For this review, take the finished solid that the model builds, in its own axes (mm). Coordinates: 2 decimals unless noted, no trailing zeros. Order: outer loops, then holes, each group sorted by start corner. A loop starts at its lowest first (then second) coordinate and runs counter-clockwise, first axis right, second up. Notation, with made-up numbers: (68, 72) -> (110, 72) arc R32 cw to (110, 105) -> close; hole circle Ø6 at (30, 80.25). An arc over 180 degrees is marked (long way). Answer as a JSON object with one key per item and string values. Group by question number.
1) Add section C-C, the plane y = -85. Write out the cut boundary in (x, z).
2) Add section A-A, the plane x = 75. Write out the cut boundary in (y, z), then the cut area to 3 significant figures.
3) Wall thickness on L1, parallel to Y at x = -75, z = -2.25; L2, parallel to X at y = -87.5, z = -1.25; L3, parallel to Y at x = 76.5, z = 4.75: over which ranges is each line inside the solid? List them lowest first.
4) For pin 1 (18 mm diameter, centred on x = 75, y = -85, fed in from +Z), flat-tipped, find the tip position at first contact; note if it passes through.
5) Add section B-B, the plane z = -4.5. Write out the cut boundary in (x, y).
from build123d import *

# Parameters (mm, degrees)
SKETCH1_W           = 250
SKETCH1_H           = 220
BOSS_EXTRUDE1_DEPTH = 8
F_14_HOLE1_D        = 14
FILLET2_R           = 20


with BuildPart() as part:
    # Sketch1 → Boss-Extrude1 (new, symmetric)
    with BuildSketch(Plane.XY):
        Rectangle(SKETCH1_W, SKETCH1_H)
    extrude(amount=BOSS_EXTRUDE1_DEPTH, both=True)

    # Ø14 Hole1 (through all)
    with Locations(Plane.XY.offset(8)):
        with Locations((-75, 85), (75, 85), (75, -85), (-75, -85)):
            Hole(F_14_HOLE1_D / 2)

    # Fillet2
    fillet2_edges = [part.edges().sort_by_distance(p)[0] for p in [
        (-125, 110, 0),
        (125, 110, 0),
        (125, -110, 0),
        (-125, -110, 0),
    ]]
    fillet(fillet2_edges, radius=FILLET2_R)


solid = part.part
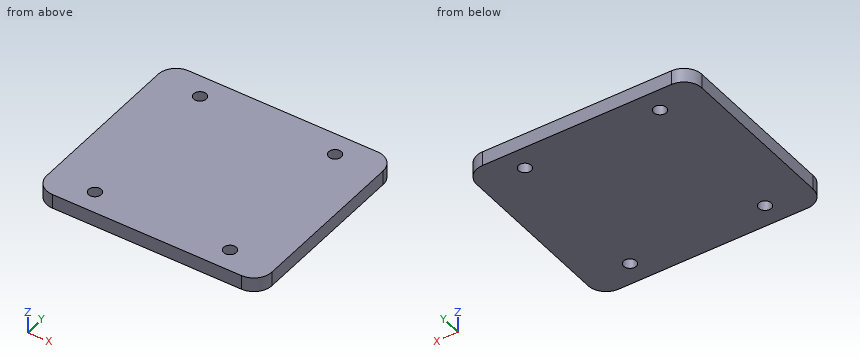
Output values:
{
 "1": {"outline": "(-125, -8) -> (-82, -8) -> (-82, 8) -> (-125, 8) -> close; (-68, -8) -> (68, -8) -> (68, 8) -> (-68, 8) -> close; (82, -8) -> (125, -8) -> (125, 8) -> (82, 8) -> close"},
 "2": {"outline": "(-110, -8) -> (-92, -8) -> (-92, 8) -> (-110, 8) -> close; (-78, -8) -> (78, -8) -> (78, 8) -> (-78, 8) -> close; (92, -8) -> (110, -8) -> (110, 8) -> (92, 8) -> close", "area": "3,070 mm²"},
 "3": {"L1": "y = -110 to -92, -78 to 78, 92 to 110", "L2": "x = -125 to -81.54, -68.46 to 68.46, 81.54 to 125", "L3": "y = -110 to -91.84, -78.16 to 78.16, 91.84 to 110"},
 "4": {"pin 1": "stops at z = 8"},
 "5": {"outline": "(-125, -90) arc R20 ccw to (-105, -110) -> (105, -110) arc R20 ccw to (125, -90) -> (125, 90) arc R20 ccw to (105, 110) -> (-105, 110) arc R20 ccw to (-125, 90) -> close; hole circle Ø14 at (-75, -85); hole circle Ø14 at (-75, 85); hole circle Ø14 at (75, -85); hole circle Ø14 at (75, 85)"}
}
